from build123d import *

# Parameters (mm, degrees)
SKETCH1_R           = 12.5
BOSS_EXTRUDE1_DEPTH = 450
SKETCH2_R           = 17.5
BOSS_EXTRUDE2_DEPTH = 50
SKETCH3_R           = 25
BOSS_EXTRUDE3_DEPTH = 12
BOSS_EXTRUDE4_START = 12
SKETCH4_R           = 25
BOSS_EXTRUDE4_DEPTH = 12
SKETCH5_R           = 10
CUT_EXTRUDE1_DEPTH  = 526.191393684


with BuildPart() as part:
    # Sketch1 → Boss-Extrude1 (new body)
    with BuildSketch(Plane.XY):
        Circle(SKETCH1_R)
    extrude(amount=BOSS_EXTRUDE1_DEPTH)

    # Sketch2 → Boss-Extrude2 (add)
    with BuildSketch(Plane(origin=(0, 0, 0), x_dir=(-1, 0, 0), z_dir=(0, 0, -1))):
        Circle(SKETCH2_R)
    extrude(amount=BOSS_EXTRUDE2_DEPTH)

    # Sketch3 → Boss-Extrude3 (add)
    with BuildSketch(Plane(origin=(0, 0, -50), x_dir=(-1, 0, 0), z_dir=(0, 0, -1))):
        Circle(SKETCH3_R)
    extrude(amount=BOSS_EXTRUDE3_DEPTH)

    # Sketch4 → Boss-Extrude4 (add)
    with BuildSketch(Plane.XY.offset(450).offset(BOSS_EXTRUDE4_START)):
        with Locations(Location((0, 0, 0), (0, 0, 180))):
            Circle(SKETCH4_R)
    extrude(amount=-BOSS_EXTRUDE4_DEPTH)

    # Sketch5 → Cut-Extrude1 (cut, through all)
    with BuildSketch(Plane.XY.offset(462)):
        Circle(SKETCH5_R)
    extrude(amount=-CUT_EXTRUDE1_DEPTH, mode=Mode.SUBTRACT)


solid = part.part
Work out the finished part from the listing and answer in its coordinate system (mm). A direction names the side the tool comes from. Give positions to 0.01 mm unless a question says otherwise; leave off trailing zeros. Loops run counter-clockwise (first coordinate to the right, second up) from the corner with the lowest first, then second, coordinate; pieces in that order, holes last. Notation, with made-up numbers: (62, 47) -> (121, 47) arc R10 cw to (121, 56) -> close; hole circle Ø5 at (57, 29). An arc over 180 degrees is marked (long way). Use a Markdown table: item, result. Add a question column.
1. Determine the mould class of faces 3 (the cylindrical face through (-23.846, 7.509, -55.916)), 4 (the flat face through (5.9, -11.5, 450)), 5 (the flat face through (0, -11, -62)) for opening direction Z: released by +Z, released by -Z, zero draft, split by the parting line, or undercut.
2. Find the intervals of material crossed by probe 1 along Z at (x, y) = (22, 3); probe 2 along Y at (x, z) = (0, 83.5); probe 3 along Z at (x, y) = (13, 3.5), in increasing order.
3. Section A-A on y = 0 is taken. Determine the outline of the cut face in (x, z), and give its area (3 significant figures).
4. For faces 1 (the cylindrical face through (11.923, 3.755, 221.85)), 2 (the flat face through (0, 11, 462)), determine the directions among +Z, -Z, +X, -X, +Y, -Y from which every point of the face is accessible in a straight line to the end or side of a thin tool.
5. Flat-ended cylindrical pins translate along their axes: pin 1 Ø8 at (x, y) = (0, 7.5) entering from +Z; pin 2 Ø3 at (x, z) = (6, 29) entering from -Y; pin 3 Ø5 at (x, z) = (14, 326) entering from +Y; pin 4 Ø1 at (x, z) = (-7, 11) entering from -Y. Find the tip coordinate at first contact, or state that the pin passes through.
6. Section C-C on z = 26.5 is taken. Determine the outline of the cut face in (x, y).
Results below:
| question | item | result |
|---|---|---|
| 1 | face 3 | zero draft |
| 1 | face 4 | undercut |
| 1 | face 5 | released by -Z |
| 2 | probe 1 | z = -62 to -50, 450 to 462 |
| 2 | probe 2 | y = -12.5 to -10, 10 to 12.5 |
| 2 | probe 3 | z = -62 to 0, 450 to 462 |
| 3 | outline | (-25, -62) -> (-10, -62) -> (-10, 462) -> (-25, 462) -> (-25, 450) -> (-12.5, 450) -> (-12.5, 0) -> (-17.5, 0) -> (-17.5, -50) -> (-25, -50) -> close; (10, -62) -> (25, -62) -> (25, -50) -> (17.5, -50) -> (17.5, 0) -> (12.5, 0) -> (12.5, 450) -> (25, 450) -> (25, 462) -> (10, 462) -> close |
| 3 | area | 3,720 mm^2 |
| 4 | face 1 | none |
| 4 | face 2 | +Z, +X, -X, +Y, -Y |
| 5 | pin 1 | stops at z = 462 |
| 5 | pin 2 | stops at y = -11.66 |
| 5 | pin 3 | stops at y = 4.9 |
| 5 | pin 4 | stops at y = -10.68 |
| 6 | outline | circle Ø25 at (0, 0); hole circle Ø20 at (0, 0) |
